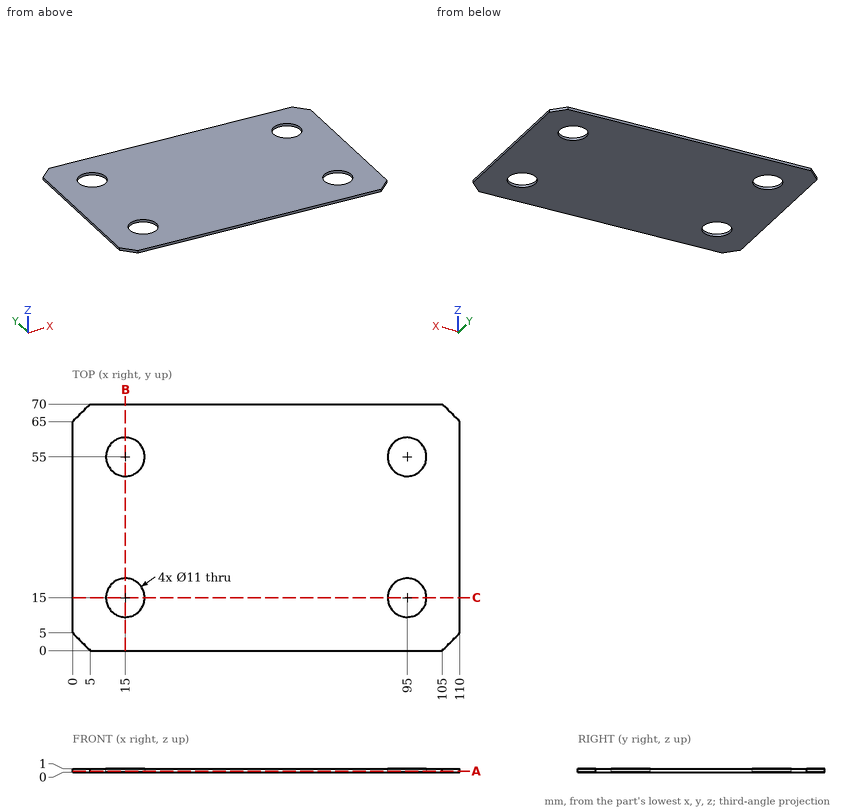
Part print with two shaded views. Sizes in mm from the minimum x, y, z corner. Round coordinates to 2 decimals unless told otherwise and drop trailing zeros. Loops run counter-clockwise (first coordinate to the right, second up) from the corner with the lowest first, then second, coordinate; pieces in that order, holes last.
Item 1: Saw through at B-B (x = 15). List the corners of the cut face in (y, z), then the cut area to 3 significant figures.
Item 2: Drill centre lines: line 1 along Y through (x, z) = (15, 0.3); line 2 along X through (y, z) = (17, 0.2); line 3 along X through (y, z) = (12, 0.3). Where is each one in solid material? Low to high.
Item 3: Saw through at C-C (y = 15). List the corners of the cut face in (x, z).
Item 4: Saw through at A-A (z = 0.25). List the corners of the cut face in (x, y).
Worked answers:
1. outline: (0, 0) - (9.5, 0) - (9.5, 1) - (0, 1) - close; (20.5, 0) - (49.5, 0) - (49.5, 1) - (20.5, 1) - close; (60.5, 0) - (70, 0) - (70, 1) - (60.5, 1) - close
1. area: 48.0 mm2
2. line 1: y = 0 to 9.5, 20.5 to 49.5, 60.5 to 70
2. line 2: x = 0 to 9.88, 20.12 to 89.88, 100.12 to 110
2. line 3: x = 0 to 10.39, 19.61 to 90.39, 99.61 to 110
3. outline: (0, 0) - (9.5, 0) - (9.5, 1) - (0, 1) - close; (20.5, 0) - (89.5, 0) - (89.5, 1) - (20.5, 1) - close; (100.5, 0) - (110, 0) - (110, 1) - (100.5, 1) - close
4. outline: (0, 5) - (5, 0) - (105, 0) - (110, 5) - (110, 65) - (105, 70) - (5, 70) - (0, 65) - close; hole circle Ø11 at (15, 15); hole circle Ø11 at (15, 55); hole circle Ø11 at (95, 15); hole circle Ø11 at (95, 55)
